Verification items for the finished model (mm, model axes). A direction names the side the tool comes from. Round coordinates to 2 decimals unless told otherwise and drop trailing zeros. Loops run counter-clockwise (first coordinate to the right, second up) from the corner with the lowest first, then second, coordinate; pieces in that order, holes last. Notation, with made-up numbers: M -26,71.25 L 26,71.25 A19 ccw 26,79.25 Z; hole C -12,39.25 d11. An arc over 180 degrees is marked long. Write item = value, one per line. Start each with the question number.
from build123d import *

# Parameters (mm, degrees)
BOSS_EXTRUDE1_DEPTH = 16


with BuildPart() as part:
    # Sketch1 → Boss-Extrude1 (new body)
    with BuildSketch(Plane.XY):
        with BuildLine():
            Line((0, 258), (15, 273))
            Line((15, 273), (120, 273))
            Line((120, 273), (120, 193.068542495))
            ThreePointArc((120, 193.068542495), (116.329931619, 181.521537111), (106.666666667, 174.212361663))
            ThreePointArc((106.666666667, 174.212361663), (80, 136.5), (106.666666667, 98.787638337))
            ThreePointArc((106.666666667, 98.787638337), (116.329931619, 91.478462889), (120, 79.931457505))
            Line((120, 79.931457505), (120, 0))
            Line((120, 0), (15, 0))
            Line((15, 0), (0, 15))
            Line((0, 15), (0, 258))
        make_face()
    extrude(amount=BOSS_EXTRUDE1_DEPTH)


solid = part.part
1. Section check A-A, the plane x = 87. Enter the section's corners in (y, z).
2. Section check C-C, the plane y = 143.5. Enter the section's corners in (x, z).
3. Section check B-B, the plane z = 8. Enter the section's corners in (x, y), and give its area (3 significant figures).
4. Thickness scan on line 1 (Y direction, x = 98.5, z = 2); line 2 (Y direction, x = 104.5, z = 4.75); line 3 (X direction, y = 109.5, z = 1). Record the ranges inside material, lowest first.
5. Mould release check, pull along Y, two halves, no side actions. Record for faces 1 (the cylindrical face through (116.23, 91.62, 7.89)), 2 (the flat face through (67, 273, 8)), 3 (the cylindrical face through (80.006, 137.189, 7.888)), 4 (the flat face through (120, 234, 8)): pulls with the +Y half, pulls with the -Y half, needs draft (parallel to the pull), parting line crosses it, or undercut.
6. Tool access check on faces 5 (the flat face through (68, 0, 8)), 6 (the cylindrical face through (116.429, 181.663, 7.888)). Record the directions out of +Z, -Z, +X, -X, +Y, -Y that give a thin tool (end or side, any length) a straight path to the whole face; none if there is none.
7. Gauge pin test, flat end, axial feed: P1, Ø4, axis at y = 98, z = 14, coming from the +X side. Record the tip position at first contact, or that the pin passes through.
8. Section check D-D, the plane y = 107. Enter the section's corners in (x, z).
Computed values:
q1.outline = M 0,0 L 113.89,0 L 113.89,16 L 0,16 Z; M 159.11,0 L 273,0 L 273,16 L 159.11,16 Z
q2.outline = M 0,0 L 80.62,0 L 80.62,16 L 0,16 Z
q3.outline = M 0,15 L 15,0 L 120,0 L 120,79.93 A20 ccw 106.67,98.79 A40 cw 106.67,174.21 A20 ccw 120,193.07 L 120,273 L 15,273 L 0,258 Z
q3.area = 29,900 mm2
q4.line_1 = 0 to 102.77, 170.23 to 273
q4.line_2 = 0 to 99.63, 173.37 to 273
q4.line_3 = 0 to 90.49
q5.face_1 = undercut
q5.face_2 = pulls with the +Y half
q5.face_3 = undercut
q5.face_4 = needs draft
q6.face_5 = +Z, -Z, +X, -X, -Y
q6.face_6 = +Z, -Z, +X
q7.P1 = 111.91
q8.outline = M 0,0 L 92.99,0 L 92.99,16 L 0,16 Z
